Verification items for the finished model (mm, model axes). Give positions to 0.01 mm unless a question says otherwise; leave off trailing zeros. Order: outer loops, then holes, each group sorted by start corner. A loop starts at its lowest first (then second) coordinate and runs counter-clockwise, first axis right, second up. Notation, with made-up numbers: M -6,15 L 4,15 A16 ccw 4,27 Z; hole C 34,-30.75 d10. An arc over 180 degrees is marked long. Answer as a JSON object with one key per item and string values.
```python
from build123d import *

# Parameters (mm, degrees)
SKETCH_1_R          = 100
EXTRUDE_1_DEPTH     = 42
CUT_EXTRUDE_1_DEPTH = 148.526268847
CUT_EXTRUDE_2_DEPTH = 138.186005117


with BuildPart() as part:
    # 草图1 → 凸台-拉伸1 (new body)
    with BuildSketch(Plane.XY):
        with Locations(Location((0, 0, 0), (0, 0, 180))):
            Circle(SKETCH_1_R)
    extrude(amount=EXTRUDE_1_DEPTH)

    # 草图2 → 切除-拉伸1 (cut, through all)
    with BuildSketch(Plane.XY.offset(42)):
        with BuildLine():
            Line((-54.258639865, 84), (54.258639865, 84))
            ThreePointArc((54.258639865, 84), (0, 100), (-54.258639865, 84))
        make_face()
        with BuildLine():
            Line((-54.258639865, -84), (54.258639865, -84))
            ThreePointArc((54.258639865, -84), (0, -100), (-54.258639865, -84))
        make_face()
    extrude(amount=-CUT_EXTRUDE_1_DEPTH, mode=Mode.SUBTRACT)

    # 草图3 → 切除-拉伸2 (cut, through all)
    with BuildSketch(Plane.XY.offset(42)):
        with BuildLine():
            Line((0, 70), (0, 84))
            Line((0, 84), (-54.258639865, 84))
            ThreePointArc((-54.258639865, 84), (-100, 0), (-54.258639865, -84))
            Line((-54.258639865, -84), (0, -84))
            Line((0, -84), (0, -70))
            ThreePointArc((0, -70), (70, 0), (0, 70))
        make_face()
    extrude(amount=-CUT_EXTRUDE_2_DEPTH, mode=Mode.SUBTRACT)


solid = part.part
```
Q1. Section check A-A on x = 49. Record the cut outline in (y, z), then the cut area to 3 significant figures.
Resolved:
{"outline": "M -84,0 L -49.99,0 L -49.99,42 L -84,42 Z; M 49.99,0 L 84,0 L 84,42 L 49.99,42 Z", "area": "2,860 mm²"}
Q2. Section check D-D on x = 38.5. Record the cut outline in (y, z).
Resolved:
{"outline": "M -84,0 L -58.46,0 L -58.46,42 L -84,42 Z; M 58.46,0 L 84,0 L 84,42 L 58.46,42 Z"}
Q3. Release check for a two-part mould opening along Y. For faces 1 (the face through (27, -84, 21)), 2 (the face through (69.983, -1.539, 21.294)), 3 (the face through (0, -77, 21)) record: +Y half, -Y half, draft (parallel to the pull), parting line (faces both ways), or undercut.
Resolved:
{"face 1": "-Y half", "face 2": "undercut", "face 3": "draft"}
Q4. Section check C-C on y = 0. Record the cut outline in (x, z), then the cut area to 3 significant figures.
Resolved:
{"outline": "M 70,0 L 100,0 L 100,42 L 70,42 Z", "area": "1,260 mm²"}
Q5. Gauge pin test, flat ends, axial feed: pin 1 Ø1 at (y, z) = (-67, 33.5) entering from +X; pin 2 Ø4 at (y, z) = (16, 5.5) entering from -X; pin 3 Ø1.5 at (y, z) = (17, 21) entering from -X. Record the tip position at first contact, or that the pin passes through.
Resolved:
{"pin 1": "stops at x = 74.68", "pin 2": "stops at x = 67.65", "pin 3": "stops at x = 67.71"}
Q6. Section check B-B on z = 4.5. Record the cut outline in (x, y), then the cut area to 3 significant figures.
Resolved:
{"outline": "M 0,-84 L 54.26,-84 A100 ccw 54.26,84 L 0,84 L 0,70 A70 cw 0,-70 Z", "area": "6,830 mm²"}
Q7. Material ranges on L1, parallel to Y at x = 48.5, z = 25.5; L2, parallel to Y at x = 5, z = 2; L3, parallel to X at y = 71, z = 32, recorded low to high.
Resolved:
{"L1": "y = -84 to -50.48, 50.48 to 84", "L2": "y = -84 to -69.82, 69.82 to 84", "L3": "x = 0 to 70.42"}
